Could you check a few things on this model? Use its own coordinates, in mm. A direction names the side the tool comes from. Round coordinates to 2 decimals unless told otherwise and drop trailing zeros. Loops run counter-clockwise (first coordinate to the right, second up) from the corner with the lowest first, then second, coordinate; pieces in that order, holes last.
from build123d import *

# Parameters (mm, degrees)
EXTRUDE_1_DEPTH     = 130
SKETCH_2_R          = 3
CUT_EXTRUDE_1_DEPTH = 20
SKETCH_9_W          = 50
SKETCH_9_H          = 55
CUT_EXTRUDE_2_DEPTH = 150
SKETCH_10_W         = 100
SKETCH_10_H         = 45
CUT_EXTRUDE_3_DEPTH = 200


with BuildPart() as part:
    # 草图1 → 凸台-拉伸1 (new body)
    with BuildSketch(Plane.XY):
        with BuildLine():
            Line((-5035.427662897, 234.022122697), (-5930.427662897, 234.022122697))
            Line((-5930.427662897, 234.022122697), (-5930.427662897, 299.022122697))
            Line((-5930.427662897, 299.022122697), (-5035.427662897, 299.022122697))
            ThreePointArc((-5035.427662897, 299.022122697), (-4802.927662897, 66.522122697), (-5035.427662897, -165.977877303))
            Line((-5035.427662897, -165.977877303), (-5235.427662897, -165.977877303))
            Line((-5235.427662897, -165.977877303), (-5235.427662897, -100.977877303))
            Line((-5235.427662897, -100.977877303), (-5035.427662897, -100.977877303))
            ThreePointArc((-5035.427662897, -100.977877303), (-4867.927662897, 66.522122697), (-5035.427662897, 234.022122697))
        make_face()
    extrude(amount=EXTRUDE_1_DEPTH)

    # 草图2 → 切除-拉伸1 (cut)
    with BuildSketch(Plane.ZY.offset(5930.427662897)):
        with Locations((6, 279.022122697)):
            Circle(SKETCH_2_R)
        with Locations((6, 254.022122697)):
            Circle(SKETCH_2_R)
        with Locations((124, 279.022122697)):
            Circle(SKETCH_2_R)
        with Locations((124, 254.022122697)):
            Circle(SKETCH_2_R)
    extrude(amount=-CUT_EXTRUDE_1_DEPTH, mode=Mode.SUBTRACT)

    # 草图9 → 切除-拉伸2 (cut)
    with BuildSketch(Plane.XY.offset(130)):
        with Locations((-5895.427662897, 266.522122697)):
            Rectangle(SKETCH_9_W, SKETCH_9_H)
    extrude(amount=-CUT_EXTRUDE_2_DEPTH, mode=Mode.SUBTRACT)

    # 草图10 → 切除-拉伸3 (cut)
    with BuildSketch(Plane.ZY.offset(5930.427662897)):
        with Locations((65, 266.522122697)):
            Rectangle(SKETCH_10_W, SKETCH_10_H)
    extrude(amount=-CUT_EXTRUDE_3_DEPTH, mode=Mode.SUBTRACT)


solid = part.part
Item 1: If we section it at A-A, the plane x = -5219: Please give me the cut outline in (y, z), then the cut area to 3 significant figures.
Results list:
outline: (-165.98, 0) - (-100.98, 0) - (-100.98, 130) - (-165.98, 130) - close; (234.02, 0) - (299.02, 0) - (299.02, 130) - (234.02, 130) - close
area: 16,900 mm2
Item 2: Will these pins go through, and if not, where does the flat tip stop? pin 1 (16.5 mm diameter, centred on y = 279, z = 34, fed in from -X); pin 2 (8 mm diameter, centred on y = 30, z = 41.5, fed in from -X); pin 3 (5 mm diameter, centred on y = 279.02, z = 124, fed in from -X); pin 4 (22.5 mm diameter, centred on x = -5799.5, y = 256, fed in from -Z).
Results list:
pin 1: stops at x = -5730.43
pin 2: stops at x = -4872.9
pin 3: stops at x = -5870.43
pin 4: stops at z = 0
Item 3: If we section it at C-C, the plane x = -4997.5: Please give me the cut outline in (y, z).
Results list:
outline: (-162.86, 0) - (-96.63, 0) - (-96.63, 130) - (-162.86, 130) - close; (229.67, 0) - (295.91, 0) - (295.91, 130) - (229.67, 130) - close
Item 4: If we section it at B-B, the plane z = 54: Please give me the cut outline in (x, y), then the cut area to 3 significant figures.
Results list:
outline: (-5930.43, 234.02) - (-5035.43, 234.02) arc R167.5 cw to (-5035.43, -100.98) - (-5235.43, -100.98) - (-5235.43, -165.98) - (-5035.43, -165.98) arc R232.5 ccw to (-5035.43, 299.02) - (-5930.43, 299.02) - (-5930.43, 289.02) - (-5920.43, 289.02) - (-5920.43, 294.02) - (-5870.43, 294.02) - (-5870.43, 289.02) - (-5730.43, 289.02) - (-5730.43, 244.02) - (-5870.43, 244.02) - (-5870.43, 239.02) - (-5920.43, 239.02) - (-5920.43, 244.02) - (-5930.43, 244.02) - close
area: 103,000 mm2
Item 5: If I drill on line 1 along Y through (x, z) = (-5925, 124); line 2 along Y through (x, z) = (-5843, 41.5); line 3 along Y through (x, z) = (-5375, 84), over which ranges is the centre line in solid material (lowest first)?
Results list:
line 1: y = 234.02 to 251.02, 257.02 to 276.02, 282.02 to 299.02
line 2: y = 234.02 to 244.02, 289.02 to 299.02
line 3: y = 234.02 to 299.02
Item 6: If we section it at D-D, the plane y = 103: Please give me the cut outline in (x, z), then the cut area to 3 significant figures.
Results list:
outline: (-4871.95, 0) - (-4805.81, 0) - (-4805.81, 130) - (-4871.95, 130) - close
area: 8,600 mm2
Item 7: For faces 1 (the cylindrical face through (-4802.984, 71.635, 64.09)), 2 (the flat face through (-5137, -100.978, 64)), 3 (the flat face through (-5870.428, 291, 66)), 4 (the flat face through (-5730.428, 267, 64)), 5 (the flat face through (-5235.428, -134, 64)), which set-ups out of +Z, -Z, +X, -X, +Y, -Y let a thin tool reach every point of the face, with its end or its side?
Results list:
face 1: +Z, -Z, +X
face 2: +Z, -Z, -X
face 3: +Z, -Z
face 4: -X
face 5: +Z, -Z, -X, -Y
Item 8: We'd pull the mould along Z, two halves only. Please class faces 6 (the flat face through (-5239, 240, 0)), 7 (the flat face through (-5801, 289.022, 64)), 8 (the flat face through (-5134, -165.978, 64)): released by +Z, released by -Z, zero draft, split by the parting line, or undercut.
Results list:
face 6: released by -Z
face 7: undercut
face 8: zero draft
